from build123d import *

# Parameters (mm, degrees)
SKETCH_1_W          = 20.5
SKETCH_1_H          = 13
EXTRUDE_1_DEPTH     = 11
CUT_EXTRUDE_1_DEPTH = 13
HOLE_WIZARD_1_D     = 7
HOLE_WIZARD_1_DEPTH = 4.4
HOLE_WIZARD_2_D     = 7
HOLE_WIZARD_2_DEPTH = 4.4
CUT_EXTRUDE_2_DEPTH = 2
CUT_EXTRUDE_3_DEPTH = 2


with BuildPart() as part:
    # 草图1 → 凸台-拉伸1 (new body)
    with BuildSketch(Plane(origin=(0, 0, 0), x_dir=(1, 0, 0), z_dir=(0, 1, 0))):
        with Locations((10.25, 6.5)):
            Rectangle(SKETCH_1_W, SKETCH_1_H)
    extrude(amount=EXTRUDE_1_DEPTH)

    # 草图2 → 切除-拉伸1 (cut)
    with BuildSketch(Plane(origin=(0, 0, 0), x_dir=(1, 0, 0), z_dir=(0, 1, 0))):
        Polygon((0, 11.8), (1, 11.8), (1, 13), (19.5, 13), (19.5, 11.8), (20.5, 11.8), (20.5, 26), (0, 26), align=None)
    extrude(amount=CUT_EXTRUDE_1_DEPTH, mode=Mode.SUBTRACT)

    # 孔1
    with Locations(Plane.XY):
        with Locations((6, 4.3)):
            Hole(HOLE_WIZARD_1_D / 2, depth=HOLE_WIZARD_1_DEPTH)

    # 孔2
    with Locations(Plane.XY):
        with Locations((14.5, 4.3)):
            Hole(HOLE_WIZARD_2_D / 2, depth=HOLE_WIZARD_2_DEPTH)

    # 草图7 → 旋转1 (revolve)
    with BuildSketch(Plane(origin=(6, 0, 0), x_dir=(0, 0, -1), z_dir=(1, 0, 0)), mode=Mode.PRIVATE) as revolve_1_sk:
        Polygon((0.4, 4.3), (0.4, 7.4), (0.8, 7.8), (4.4, 7.8), (4.4, 4.3), align=None)
    revolve(revolve_1_sk.sketch.rotate(Axis((6, 4.3, -4.4), (0, 0, 1)), 270), axis=Axis((6, 4.3, -4.4), (0, 0, 1)))

    # 草图8 → 旋转2 (revolve)
    with BuildSketch(Plane(origin=(14.5, 0, 0), x_dir=(0, 0, -1), z_dir=(1, 0, 0)), mode=Mode.PRIVATE) as revolve_2_sk:
        Polygon((0.4, 4.3), (0.4, 7.4), (0.8, 7.8), (4.4, 7.8), (4.4, 4.3), align=None)
    revolve(revolve_2_sk.sketch.rotate(Axis((14.5, 4.3, -4.4), (0, 0, 1)), 270), axis=Axis((14.5, 4.3, -4.4), (0, 0, 1)))

    # 草图9 → 切除-拉伸2 (cut)
    with BuildSketch(Plane.XY.offset(-0.4)):
        Polygon((4.5, 5.166025404), (4.5, 3.433974596), (6, 2.567949192), (7.5, 3.433974596), (7.5, 5.166025404), (6, 6.032050808), align=None)
    extrude(amount=-CUT_EXTRUDE_2_DEPTH, mode=Mode.SUBTRACT)

    # 草图10 → 切除-拉伸3 (cut)
    with BuildSketch(Plane.XY.offset(-0.4)):
        Polygon((13, 3.433974596), (14.5, 2.567949192), (16, 3.433974596), (16, 5.166025404), (14.5, 6.032050808), (13, 5.166025404), align=None)
    extrude(amount=-CUT_EXTRUDE_3_DEPTH, mode=Mode.SUBTRACT)


solid = part.part
Geometry check sheet. Reference: the model listing, model coordinates, mm. A direction names the side the tool comes from. Give positions to 0.01 mm unless a question says otherwise; leave off trailing zeros. Write each loop counter-clockwise with the first axis right and the second up, starting at its lowest first coordinate (ties: lowest second). Pieces come first, ordered by that corner, then holes. Notation, with made-up numbers: M 39,57.25 L 56,57.25 A17 cw 56,70.25 Z; hole C -14.75,29 d11. An arc over 180 degrees is marked long. One line per question, with ' | ' between items.
1. Scan lines: line 1 along X through (y, z) = (4.3, -0.15); line 2 along Y through (x, z) = (6, -0.25); line 3 along Z through (x, y) = (14.5, 6). Record each from-to range of solid material in increasing order. Write a range as from..to.
Ans:
line 1: 0..2.5, 9.5..11, 18..20.5 | line 2: 0..0.8, 7.8..11 | line 3: -13..-2.4
2. Set-up check for faces 4 (the face through (0.5, 5.4, -11.8)), 5 (the face through (5.24, 3.007, -1.386)), 6 (the face through (20.5, 5, -6)): record each of +Z, -Z, +X, -X, +Y, -Y from which the full face is reachable in a straight line by a thin tool's end or side.
Ans:
face 4: -Z, -X, +Y, -Y | face 5: +Z | face 6: +Z, -Z, +X, +Y, -Y
3. Mould release check, pull along X, two halves, no side actions. Record for faces 1 (the face through (19.5, 5, -12)), 2 (the face through (20, 5, -11.8)), 3 (the face through (5, 6, -0.4)): released by +X, released by -X, zero draft, split by the parting line, or undercut.
Ans:
face 1: released by +X | face 2: zero draft | face 3: undercut
4. Cross-section at A-A (y = 4.3). Enter the section's corners in (x, z), plus the area to 3 significant figures.
Ans:
outline: M 0,-11.8 L 1,-11.8 L 1,-13 L 19.5,-13 L 19.5,-11.8 L 20.5,-11.8 L 20.5,0 L 18,0 L 18,-0.8 L 17.6,-0.4 L 16,-0.4 L 16,-2.4 L 13,-2.4 L 13,-0.4 L 11.4,-0.4 L 11,-0.8 L 11,0 L 9.5,0 L 9.5,-0.8 L 9.1,-0.4 L 7.5,-0.4 L 7.5,-2.4 L 4.5,-2.4 L 4.5,-0.4 L 2.9,-0.4 L 2.5,-0.8 L 2.5,0 L 0,0 Z | area: 246 mm2
5. Gauge pin test, flat ends, axial feed: pin 1 (0.8 mm diameter, centred on x = 20, y = 7, fed in from -Z); pin 2 (3 mm diameter, centred on x = 5, y = 5, fed in from +Z); pin 3 (0.9 mm diameter, centred on x = 6.5, y = 5, fed in from +Z). Record the tip position at first contact, or that the pin passes through.
Ans:
pin 1: z = -11.8 | pin 2: z = -0.4 | pin 3: z = -2.4
